from build123d import *

# Parameters (mm, degrees)
BOSS_EXTRUDE1_DEPTH      = 700
BOSS_EXTRUDE1_DEPTH_BACK = 1259
SKETCH1_W                = 120
SKETCH1_H                = 120
SKETCH2_W                = 20.088480041
SKETCH2_H                = 120
CUT_EXTRUDE1_DEPTH       = 2985
BOSS_EXTRUDE2_START      = -750
SKETCH3_W                = 119.911519959
SKETCH3_H                = 140
BOSS_EXTRUDE2_DEPTH      = 10
BOSS_EXTRUDE3_START      = -300
SKETCH4_W                = 139.911519959
SKETCH4_H                = 160
BOSS_EXTRUDE3_DEPTH      = 10
SKETCH5_R                = 5
CUT_EXTRUDE2_DEPTH       = 10


with BuildPart() as part:
    # Sketch1 → Boss-Extrude1 (new, two sides: drawn at the far end of the back side and taken through both)
    with BuildSketch(Plane.XY.offset(-BOSS_EXTRUDE1_DEPTH_BACK)):
        with Locations((0, 160)):
            Rectangle(SKETCH1_W, SKETCH1_H)
    extrude(amount=BOSS_EXTRUDE1_DEPTH + BOSS_EXTRUDE1_DEPTH_BACK)

    # Sketch2 → Cut-Extrude1 (cut)
    with BuildSketch(Plane.XY.offset(700)):
        with Locations((-49.95575998, 160)):
            Rectangle(SKETCH2_W, SKETCH2_H)
    extrude(amount=-CUT_EXTRUDE1_DEPTH, mode=Mode.SUBTRACT)

    # Sketch3 → Boss-Extrude2 (add)
    with BuildSketch(Plane(origin=(0, 0, -1259), x_dir=(-1, 0, 0), z_dir=(0, 0, -1)).offset(BOSS_EXTRUDE2_START)):
        with Locations((-10.04424002, 160)):
            Rectangle(SKETCH3_W, SKETCH3_H)
    extrude(amount=BOSS_EXTRUDE2_DEPTH)

    # Sketch4 → Boss-Extrude3 (add)
    with BuildSketch(Plane.XY.offset(700).offset(BOSS_EXTRUDE3_START)):
        with Locations((10.04424002, 160)):
            Rectangle(SKETCH4_W, SKETCH4_H)
    extrude(amount=BOSS_EXTRUDE3_DEPTH)

    # Sketch5 → Cut-Extrude2 (cut)
    with BuildSketch(Plane.XY.offset(410)):
        with Locations((70, 230)):
            Circle(SKETCH5_R)
        with Locations((70, 90)):
            Circle(SKETCH5_R)
        with Locations((-49.911519959, 90)):
            Circle(SKETCH5_R)
        with Locations((-49.911519959, 230)):
            Circle(SKETCH5_R)
    extrude(amount=-CUT_EXTRUDE2_DEPTH, mode=Mode.SUBTRACT)


solid = part.part
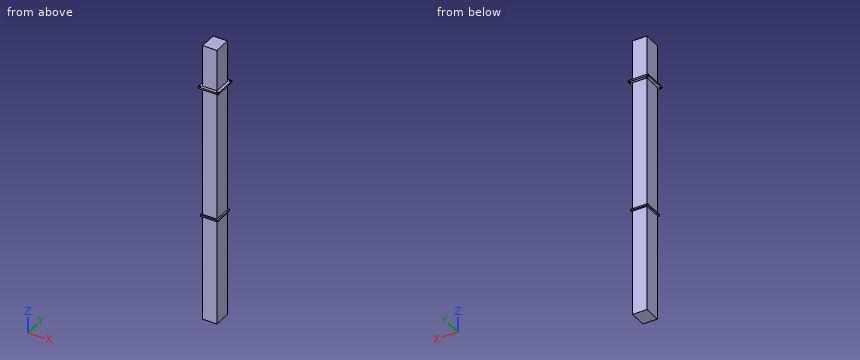
Part model, mm, in its own coordinate system. Round coordinates to 2 decimals unless told otherwise and drop trailing zeros. Loops run counter-clockwise (first coordinate to the right, second up) from the corner with the lowest first, then second, coordinate; pieces in that order, holes last. Notation, with made-up numbers: (41, 71.25) - (47, 71.25) arc R6 cw to (47, 77.25) - close; hole circle Ø3 at (33.5, -13.75). An arc over 180 degrees is marked (long way). Answer as a JSON object with one key per item and string values.
Item 1: Band-saw the part on A-A on y = 131.5. List the corners of the cut face in (x, z).
Output:
{"outline": "(-59.91, 400) - (-39.91, 400) - (-39.91, -509) - (-49.91, -509) - (-49.91, -519) - (-39.91, -519) - (-39.91, -1259) - (60, -1259) - (60, -519) - (70, -519) - (70, -509) - (60, -509) - (60, 400) - (80, 400) - (80, 410) - (60, 410) - (60, 700) - (-39.91, 700) - (-39.91, 410) - (-59.91, 410) - close"}
Item 2: Band-saw the part on B-B on x = 38.5. List the corners of the cut face in (y, z), plus the area to 3 significant figures.
Output:
{"outline": "(80, 400) - (100, 400) - (100, -509) - (90, -509) - (90, -519) - (100, -519) - (100, -1259) - (220, -1259) - (220, -519) - (230, -519) - (230, -509) - (220, -509) - (220, 400) - (240, 400) - (240, 410) - (220, 410) - (220, 700) - (100, 700) - (100, 410) - (80, 410) - close", "area": "236,000 mm2"}
Item 3: Band-saw the part on C-C on z = -143.5. List the corners of the cut face in (x, y).
Output:
{"outline": "(-39.91, 100) - (60, 100) - (60, 220) - (-39.91, 220) - close"}
Item 4: Pin check, flat tips, straight feed: pin 1 (12 mm diameter, centred on y = 103.5, z = -566, fed in from -X); pin 2 (8 mm diameter, centred on x = 2, z = -632, fed in from -Y); pin 3 (8 mm diameter, centred on x = -49.91, y = 230, fed in from -Z). Stop position of each tip, or through.
Output:
{"pin 1": "x = -39.91", "pin 2": "y = 100", "pin 3": "z = -519"}
Item 5: Wall check: L1, parallel to Y at x = 70, z = 405; L2, parallel to Z at x = 62.5, y = 170; L3, parallel to Y at x = -36.5, z = -594.5. Give the ranges that are in metal, low to high.
Output:
{"L1": "80 to 85, 95 to 225, 235 to 240", "L2": "-519 to -509, 400 to 410", "L3": "100 to 220"}
